from build123d import *

# Parameters (mm, degrees)
SKETCH_1_W          = 220
SKETCH_1_H          = 121
EXTRUDE_1_DEPTH     = 2.5
CUT_EXTRUDE_1_DEPTH = 164.603178453
SKETCH_5_W          = 6
SKETCH_5_H          = 8
CUT_EXTRUDE_2_DEPTH = 159.13680786
FILLET_1_R          = 5
FILLET_2_R          = 3
CHAMFER_1_SIZE      = 0.5


with BuildPart() as part:
    # 草图1 → 凸台-拉伸1 (new, symmetric)
    with BuildSketch(Plane.XY):
        with Locations((0, 60.5)):
            Rectangle(SKETCH_1_W, SKETCH_1_H)
    extrude(amount=EXTRUDE_1_DEPTH, both=True)

    # 草图4 → 切除-拉伸1 (cut, through all)
    with BuildSketch(Plane.XY.offset(2.5)):
        with BuildLine():
            Line((-94, 66), (-110, 66))
            Line((-110, 66), (-110, 125.2))
            Line((-110, 125.2), (110, 125.2))
            Line((110, 125.2), (110, 66))
            Line((110, 66), (94, 66))
            Line((94, 66), (94, 89.205740869))
            ThreePointArc((94, 89.205740869), (91.081973046, 97.760848899), (83.544303797, 102.749666097))
            ThreePointArc((83.544303797, 102.749666097), (0, 113.5), (-83.544303797, 102.749666097))
            ThreePointArc((-83.544303797, 102.749666097), (-91.081973046, 97.760848899), (-94, 89.205740869))
            Line((-94, 89.205740869), (-94, 66))
        make_face()
    extrude(amount=-CUT_EXTRUDE_1_DEPTH, mode=Mode.SUBTRACT)

    # 草图5 → 切除-拉伸2 (cut, through all)
    with BuildSketch(Plane.XY.offset(2.5)):
        with Locations((-107, 53.5)):
            Rectangle(SKETCH_5_W, SKETCH_5_H)
        with Locations((107, 53.5)):
            Rectangle(SKETCH_5_W, SKETCH_5_H)
    extrude(amount=-CUT_EXTRUDE_2_DEPTH, mode=Mode.SUBTRACT)

    # 圆角1
    fillet_1_edges = [part.edges().sort_by_distance(p)[0] for p in [
        (-110, 66, 0),
        (110, 66, 0),
        (110, 0, 0),
        (-110, 0, 0),
    ]]
    fillet(fillet_1_edges, radius=FILLET_1_R)

    # 圆角2
    fillet_2_edges = [part.edges().sort_by_distance(p)[0] for p in [
        (-94, 66, 0),
        (94, 66, 0),
        (-104, 57.5, 0),
        (-104, 49.5, 0),
        (104, 49.5, 0),
        (104, 57.5, 0),
    ]]
    fillet(fillet_2_edges, radius=FILLET_2_R)

    # 倒角1
    chamfer_1_edges = [part.edges().sort_by_distance(p)[0] for p in [
        (-94, 79.102870434, 2.5),
        (101, 66, 2.5),
        (-104, 53.5, 2.5),
        (-108.5, 57.5, 2.5),
        (108.5, 49.5, 2.5),
        (104, 53.5, 2.5),
        (-94.878679656, 66.878679656, 2.5),
        (94.878679656, 66.878679656, 2.5),
        (-104.878679656, 50.378679656, 2.5),
        (-104.878679656, 56.621320344, 2.5),
        (104.878679656, 50.378679656, 2.5),
        (104.878679656, 56.621320344, 2.5),
        (-91.081973046, 97.760848899, 2.5),
        (0, 113.5, 2.5),
        (91.081973046, 97.760848899, 2.5),
        (94, 79.102870434, 2.5),
        (-110, 27.25, 2.5),
        (-108.5, 49.5, 2.5),
        (110, 59.25, 2.5),
        (108.5, 57.5, 2.5),
        (-101, 66, 2.5),
        (-110, 59.25, 2.5),
        (0, 0, 2.5),
        (110, 27.25, 2.5),
        (108.535533906, 1.464466094, 2.5),
        (-108.535533906, 1.464466094, 2.5),
        (108.535533906, 64.535533906, 2.5),
        (-108.535533906, 64.535533906, 2.5),
    ]]
    chamfer(chamfer_1_edges, length=CHAMFER_1_SIZE)


solid = part.part
Model file for the job. Use its own axes, mm. A direction names the side the tool comes from. Coordinates: 2 decimals unless noted, no trailing zeros. Order: outer loops, then holes, each group sorted by start corner. A loop starts at its lowest first (then second) coordinate and runs counter-clockwise, first axis right, second up. Notation, with made-up numbers: (4.5, 22.5) -> (48.5, 22.5) arc R22 cw to (48.5, 58.5) -> close; hole circle Ø6 at (-26.5, 85.5). An arc over 180 degrees is marked (long way). Return JSON: item names as keys, results as strings. Group by question number.
Item 1: Tool access for faces 1 (the flat face through (94, 79, 0)), 2 (the flat face through (-2, 58, -2.5)), 3 (the flat face through (-94, 79, 0)): list every direction of +Z, -Z, +X, -X, +Y, -Y with a clear straight run to the whole face (end or side of a thin tool).
Item 2: Saw through at A-A on z = 0.8. Write the cut outline in (x, y).
Item 3: Flat gauge pins, fed straight in: P1, Ø1.3, axis at x = 101, z = 0.5, coming from the +Y side; P2, Ø0.6, axis at y = 53.5, z = 0, coming from the -X side; P3, Ø3, axis at y = 67, z = 2, coming from the -X side. Where does each tip first touch, or does it go through?
Item 4: Saw through at B-B on y = 73.5. Write the cut outline in (x, z), then the cut area to 3 significant figures.
Item 5: Wall check: line 1 along X through (y, z) = (87.5, 1.6); line 2 along Y through (x, z) = (-1.5, 0.15); line 3 along Y through (x, z) = (-16, -2.15). Give the ranges that are in metal, low to high. Write a range as [from, to].
Values found:
{
 "1": {"face 1": "+Z, -Z, +X, +Y", "face 2": "-Z, +X, -X, +Y, -Y", "face 3": "+Z, -Z, -X, +Y"},
 "2": {"outline": "(-110, 5) arc R5 ccw to (-105, 0) -> (105, 0) arc R5 ccw to (110, 5) -> (110, 49.5) -> (107, 49.5) arc R3 cw to (104, 52.5) -> (104, 54.5) arc R3 cw to (107, 57.5) -> (110, 57.5) -> (110, 61) arc R5 ccw to (105, 66) -> (97, 66) arc R3 cw to (94, 69) -> (94, 89.21) arc R14 ccw to (83.54, 102.75) arc R330 ccw to (-83.54, 102.75) arc R14 ccw to (-94, 89.21) -> (-94, 69) arc R3 cw to (-97, 66) -> (-105, 66) arc R5 ccw to (-110, 61) -> (-110, 57.5) -> (-107, 57.5) arc R3 cw to (-104, 54.5) -> (-104, 52.5) arc R3 cw to (-107, 49.5) -> (-110, 49.5) -> close"},
 "3": {"P1": "stops at y = 66", "P2": "stops at x = -104", "P3": "stops at x = -107.18"},
 "4": {"outline": "(-94, -2.5) -> (94, -2.5) -> (94, 2) -> (93.5, 2.5) -> (-93.5, 2.5) -> (-94, 2) -> close", "area": "940 mm2"},
 "5": {"line 1": "x = [-94, 94]", "line 2": "y = [0, 113.5]", "line 3": "y = [0, 113.11]"}
}
